from build123d import *

# Parameters (mm, degrees)
EXTRUDE_1_DEPTH     = 1000
SHELL_1_T           = -2
SKETCH_3_W          = 400
SKETCH_3_H          = 800
CUT_EXTRUDE_1_DEPTH = 30
SKETCH_4_W          = 404
SKETCH_4_H          = 804
SKETCH_4_W_2        = 400
SKETCH_4_H_2        = 800
EXTRUDE_2_DEPTH     = 34
EXTRUDE_3_DEPTH     = 2
SKETCH_6_W          = 600
SKETCH_6_H          = 200
CUT_EXTRUDE_2_DEPTH = 1044
SKETCH_10_W         = 600
SKETCH_10_H         = 425
CUT_EXTRUDE_4_DEPTH = 1005
SKETCH_11_W         = 28
SKETCH_11_H         = 998
EXTRUDE_5_DEPTH     = 2
SKETCH_12_W         = 498.34314575
SKETCH_12_H         = 30
SKETCH_12_W_2       = 28
SKETCH_12_H_2       = 72.171572875
EXTRUDE_6_DEPTH     = 2
SKETCH_13_R         = 3
CUT_EXTRUDE_5_DEPTH = 1280
SKETCH_14_R         = 3
CUT_EXTRUDE_6_DEPTH = 10
SKETCH_15_R         = 3
CUT_EXTRUDE_7_DEPTH = 28
SKETCH_16_R         = 3
CUT_EXTRUDE_8_DEPTH = 10


with BuildPart() as part:
    # 草图1 → 凸台-拉伸1 (new body)
    with BuildSketch(Plane.XY):
        Polygon((0, 700), (50, 750), (550, 750), (600, 700), (600, 0), (0, 0), align=None)
    extrude(amount=EXTRUDE_1_DEPTH)

    # 抽壳1
    shell_1_openings = [part.faces().sort_by_distance(p)[0] for p in [
        (300, 372.998137803, 1000),
    ]]
    offset(amount=SHELL_1_T, openings=shell_1_openings, kind=Kind.INTERSECTION)

    # 草图3 → 切除-拉伸1 (cut)
    with BuildSketch(Plane(origin=(0, 750, 0), x_dir=(1, 0, 0), z_dir=(0, 1, 0))):
        with Locations((300, -550)):
            Rectangle(SKETCH_3_W, SKETCH_3_H)
    extrude(amount=-CUT_EXTRUDE_1_DEPTH, mode=Mode.SUBTRACT)

    # 草图4 → 凸台-拉伸2 (add)
    with BuildSketch(Plane(origin=(0, 750, 0), x_dir=(1, 0, 0), z_dir=(0, 1, 0))):
        with Locations((300, -550)):
            Rectangle(SKETCH_4_W, SKETCH_4_H)
        with Locations((300, -550)):
            Rectangle(SKETCH_4_W_2, SKETCH_4_H_2, mode=Mode.SUBTRACT)
    extrude(amount=-EXTRUDE_2_DEPTH)

    # 草图5 → 凸台-拉伸3 (add)
    with BuildSketch(Plane.XZ.offset(-716)):
        Polygon((128, 178), (472, 178), (472, 922), (128, 922), (100, 922), (100, 950), (500, 950), (500, 150), (100, 150), (100, 178), align=None)
    extrude(amount=-EXTRUDE_3_DEPTH)

    # 草图6 → 切除-拉伸2 (cut)
    with BuildSketch(Plane(origin=(0, 0, 0), x_dir=(-1, 0, 0), z_dir=(0, 0, -1))):
        with Locations((-300, 100)):
            Rectangle(SKETCH_6_W, SKETCH_6_H)
    extrude(amount=-CUT_EXTRUDE_2_DEPTH, mode=Mode.SUBTRACT)

    # 草图10 → 切除-拉伸4 (cut)
    with BuildSketch(Plane(origin=(0, 0, 0), x_dir=(-1, 0, 0), z_dir=(0, 0, -1))):
        with Locations((-300, 412.5)):
            Rectangle(SKETCH_10_W, SKETCH_10_H)
    extrude(amount=-CUT_EXTRUDE_4_DEPTH, mode=Mode.SUBTRACT)

    # 草图11 → 凸台-拉伸5 (add)
    with BuildSketch(Plane.XZ.offset(-625)):
        with Locations((16, 501)):
            Rectangle(SKETCH_11_W, SKETCH_11_H)
        with Locations((584, 501)):
            Rectangle(SKETCH_11_W, SKETCH_11_H)
    extrude(amount=-EXTRUDE_5_DEPTH)

    # 草图12 → 凸台-拉伸6 (add)
    with BuildSketch(Plane.XY.offset(1000)):
        with Locations((300, 733)):
            Rectangle(SKETCH_12_W, SKETCH_12_H)
        with Locations((16, 663.085786438)):
            Rectangle(SKETCH_12_W_2, SKETCH_12_H_2)
        with Locations((584, 663.085786438)):
            Rectangle(SKETCH_12_W_2, SKETCH_12_H_2)
    extrude(amount=-EXTRUDE_6_DEPTH)

    # 草图13 → 切除-拉伸5 (cut)
    with BuildSketch(Plane.XY.offset(1000)):
        with Locations((585, 665)):
            Circle(SKETCH_13_R)
        with Locations((15, 665)):
            Circle(SKETCH_13_R)
    extrude(amount=-CUT_EXTRUDE_5_DEPTH, mode=Mode.SUBTRACT)

    # 草图14 → 切除-拉伸6 (cut)
    with BuildSketch(Plane.XZ.offset(-625)):
        with Locations((15, 970)):
            Circle(SKETCH_14_R)
        with Locations((15, 670)):
            Circle(SKETCH_14_R)
        with Locations(Location((585, 120, 0), (0, 0, 270))):
            Circle(SKETCH_14_R)
        with Locations((15, 370)):
            Circle(SKETCH_14_R)
        with Locations(Location((585, 370, 0), (0, 0, 270))):
            Circle(SKETCH_14_R)
        with Locations((15, 120)):
            Circle(SKETCH_14_R)
        with Locations(Location((585, 670, 0), (0, 0, 270))):
            Circle(SKETCH_14_R)
        with Locations(Location((585, 970, 0), (0, 0, 270))):
            Circle(SKETCH_14_R)
    extrude(amount=-CUT_EXTRUDE_6_DEPTH, mode=Mode.SUBTRACT)

    # 草图15 → 切除-拉伸7 (cut)
    with BuildSketch(Plane.XY.offset(1000)):
        with Locations((150.828427125, 735)):
            Circle(SKETCH_15_R)
        with Locations((449.171572875, 735)):
            Circle(SKETCH_15_R)
    extrude(amount=-CUT_EXTRUDE_7_DEPTH, mode=Mode.SUBTRACT)

    # 草图16 → 切除-拉伸8 (cut)
    with BuildSketch(Plane(origin=(0, 0, 0), x_dir=(-1, 0, 0), z_dir=(0, 0, -1))):
        with Locations((-450, 735)):
            Circle(SKETCH_16_R)
        with Locations((-150, 734.726066428)):
            Circle(SKETCH_16_R)
    extrude(amount=-CUT_EXTRUDE_8_DEPTH, mode=Mode.SUBTRACT)


solid = part.part
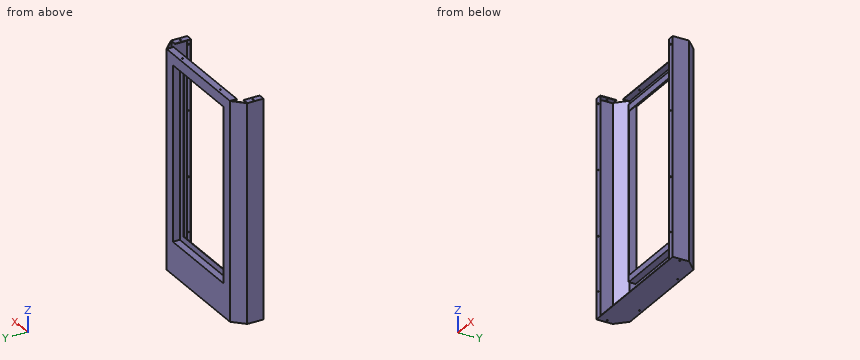
Build history of the part. All positions in model axes, mm. Coordinates: 2 decimals unless noted, no trailing zeros. Write each loop counter-clockwise with the first axis right and the second up, starting at its lowest first coordinate (ties: lowest second). Pieces come first, ordered by that corner, then holes.
(1) Pin check, flat tips, straight feed: pin 1 Ø9.5 at (y, z) = (729, 390.5) entering from +X; pin 2 Ø7 at (x, y) = (585, 665) entering from +Z; pin 3 Ø16 at (y, z) = (729.5, 700.5) entering from -X; pin 4 Ø6 at (x, z) = (206, 118) entering from -Y. Stop position of each tip, or through.
(2) Cut at A-A on z = 782. List the corners of the cut face in (x, y).
(3) Drill centre lines: line 1 (X direction, y = 626.25, z = 370); line 2 (Z direction, x = 15, y = 625.7); line 3 (X direction, y = 665, z = 1.25). Where is each one in solid material? Low to high.
(4) Cut at B-B on x = 194.5. List the corners of the cut face in (y, z).
Working result:
1. pin 1: stops at x = 575.75
1. pin 2: stops at z = 1000
1. pin 3: stops at x = 21.5
1. pin 4: stops at y = 748
2. outline: (0, 625) - (30, 625) - (30, 627) - (2, 627) - (2, 699.17) - (50.83, 748) - (98, 748) - (98, 716) - (100, 716) - (100, 750) - (50, 750) - (0, 700) - close; (472, 716) - (502, 716) - (502, 748) - (549.17, 748) - (598, 699.17) - (598, 627) - (570, 627) - (570, 625) - (600, 625) - (600, 700) - (550, 750) - (500, 750) - (500, 718) - (472, 718) - close
3. line 1: x = 0 to 12, 18 to 30, 570 to 582, 588 to 600
3. line 2: z = 0 to 117, 123 to 367, 373 to 667, 673 to 967, 973 to 1000
3. line 3: x = 0 to 12, 18 to 582, 588 to 600
4. outline: (625, 0) - (750, 0) - (750, 150) - (718, 150) - (718, 178) - (716, 178) - (716, 148) - (748, 148) - (748, 2) - (625, 2) - close; (716, 922) - (718, 922) - (718, 950) - (750, 950) - (750, 1000) - (718, 1000) - (718, 998) - (748, 998) - (748, 952) - (716, 952) - close
